```python
from build123d import *


with BuildPart() as part:
    # 草图1 → 旋转1 (revolve)
    with BuildSketch(Plane.XY, mode=Mode.PRIVATE) as revolve_1_sk:
        Polygon((-4, 32.5), (-17.6, 32.5), (-17.6, 22.5), (-24, 22.5), (-24, 0), (-20, 0), (-20, 15), (-4, 20.6), align=None)
    revolve(revolve_1_sk.sketch.rotate(Axis((0, 61.8, 0), (0, -1, 0)), 270), axis=Axis((0, 61.8, 0), (0, -1, 0)))


solid = part.part
```
Input: part model. Units: mm. Frame: model coordinates. A direction names the side the tool comes from. Give positions to 0.01 mm unless a question says otherwise; leave off trailing zeros. Order: outer loops, then holes, each group sorted by start corner. A loop starts at its lowest first (then second) coordinate and runs counter-clockwise, first axis right, second up. Notation, with made-up numbers: M 68.5,76 L 82.5,76 A20 cw 82.5,95 Z; hole C 11,-38.75 d3. An arc over 180 degrees is marked long. One line per question, with ' | ' between items. Start each with the question number.
1. Material intervals for probe 1 along X at (y, z) = (25.5, 0); probe 2 along Y at (x, z) = (-12.5, -16.5); probe 3 along Z at (x, y) = (-5, 14), sorted ascending. Write a range as [from, to].
2. Section query D-D (y = 29.5). Return the cut outline in (x, z), and give its area (3 significant figures).
3. Section query C-C (y = 9). Return the cut outline in (x, z), and give its area (3 significant figures).
4. Section query A-A (x = 0). Return the cut outline in (y, z).
5. Section query B-B (z = 0). Return the cut outline in (x, y), and give its area (3 significant figures).
6. First-contact query: pin 1 Ø1 at (x, y) = (-13.5, 4) entering from +Z; pin 2 Ø1.5 at (x, y) = (9.5, 28) entering from +Z; pin 3 Ø8 at (y, z) = (22.5, -19) entering from +X (3 decimals). Flat tips, straight axial feed; report the tip coordinate or a pass-through.
7. Access query for faces 5 (the face through (3.905, 26.633, -0.867)), 6 (the face through (-13, 22.5, 13)). Directions: +Z, -Z, +X, -X, +Y, -Y. A direction counts if a zero-diameter tool reaches every point of the face in a straight line with its end or side. Return the directions, or none.
8. Pull-direction query (Z, two-part tool) for faces 1 (the face through (-17.45, 27.43, -2.29)), 2 (the face through (-4.2, 32.5, 0.2)), 3 (the face through (-1.435, 20.328, 4.556)), 4 (the face through (19.524, 7.605, -4.336)); classes: released by +Z, released by -Z, zero draft, split by the parting line, or undercut.
Here are the results:
1) probe 1: [-17.6, -4], [4, 17.6] | probe 2: [0, 22.5] | probe 3: [-23.47, -19.36], [19.36, 23.47]
2) outline: C 0,0 d35.2; hole C 0,0 d8 | area: 923 mm²
3) outline: C 0,0 d48; hole C 0,0 d40 | area: 553 mm²
4) outline: M 0,-24 L 22.5,-24 L 22.5,-17.6 L 32.5,-17.6 L 32.5,-4 L 20.6,-4 L 15,-20 L 0,-20 Z; M 0,20 L 15,20 L 20.6,4 L 32.5,4 L 32.5,17.6 L 22.5,17.6 L 22.5,24 L 0,24 Z
5) outline: M -24,0 L -20,0 L -20,15 L -4,20.6 L -4,32.5 L -17.6,32.5 L -17.6,22.5 L -24,22.5 Z; M 4,20.6 L 20,15 L 20,0 L 24,0 L 24,22.5 L 17.6,22.5 L 17.6,32.5 L 4,32.5 Z | area: 602 mm²
6) pin 1: z = 20.17 | pin 2: z = 15.27 | pin 3: x = 18.735
7) face 5: +Y, -Y | face 6: +Y
8) face 1: split by the parting line | face 2: zero draft | face 3: undercut | face 4: undercut
